from build123d import *

# Parameters (mm, degrees)
SKETCH_1_W              = 50
SKETCH_1_H              = 320
EXTRUDE_1_DEPTH         = 7.5
EXTRUDE_2_DEPTH         = 52.5
EXTRUDE_2_DEPTH_BACK    = 7.5
SKETCH_2_R              = 25
SKETCH_3_R              = 15
CUT_EXTRUDE_1_DEPTH     = 197.086715511
HOLE_WIZARD_12_0_12_1_D = 12


with BuildPart() as part:
    # 草图1 → 凸台-拉伸1 (new, symmetric)
    with BuildSketch(Plane(origin=(0, 0, 0), x_dir=(0, 0, -1), z_dir=(1, 0, 0))):
        Rectangle(SKETCH_1_W, SKETCH_1_H)
    extrude(amount=EXTRUDE_1_DEPTH, both=True)

    # 草图2 → 凸台-拉伸2 (add, two sides: drawn at the far end of the back side and taken through both)
    with BuildSketch(Plane(origin=(0, 0, 0), x_dir=(0, 0, -1), z_dir=(1, 0, 0)).offset(-EXTRUDE_2_DEPTH_BACK)):
        with Locations((0, 160)):
            Circle(SKETCH_2_R)
    extrude(amount=EXTRUDE_2_DEPTH + EXTRUDE_2_DEPTH_BACK)

    # 草图3 → 切除-拉伸1 (cut, through all)
    with BuildSketch(Plane(origin=(52.5, 0, 0), x_dir=(0, 0, -1), z_dir=(1, 0, 0))):
        with Locations((0, 160)):
            Circle(SKETCH_3_R)
    extrude(amount=-CUT_EXTRUDE_1_DEPTH, mode=Mode.SUBTRACT)

    # Ø12.0 (12) 直径孔1 (through all)
    with Locations(Plane.ZY.offset(7.5)):
        with Locations((0, 22), (0, -148)):
            Hole(HOLE_WIZARD_12_0_12_1_D / 2)


solid = part.part
The model under review builds one solid part; all positions refer to its coordinate system, in mm. A direction names the side the tool comes from. Round coordinates to 2 decimals unless told otherwise and drop trailing zeros. Write each loop counter-clockwise with the first axis right and the second up, starting at its lowest first coordinate (ties: lowest second). Pieces come first, ordered by that corner, then holes. Notation, with made-up numbers: M -16,86.25 L 3,86.25 A8 ccw 3,94.25 Z; hole C 63.5,-17.75 d6. An arc over 180 degrees is marked long. Answer as CSV lines item,"result". Start each with the question number.
Q1. Consider section A-A, the plane z = 0. Give the boundary of the cut face in (x, y).
Q2. Tool access review of faces 1 (the face through (22.08, 184.787, 3.255)), 2 (the face through (0.105, 16.143, 1.301)): name each direction out of +Z, -Z, +X, -X, +Y, -Y from which nothing blocks a thin tool from reaching the whole face with its end or side.
Q3. Clearance check with flat-ended pins moving along their axes: P1, Ø1, axis at x = 28, z = -3.5, coming from the +Y side; P2, Ø4, axis at y = 74, z = 8.5, coming from the +X side; P3, Ø5, axis at x = 22, z = -13.5, coming from the +Y side; P4, Ø15.5, axis at y = -148, z = 0, coming from the -X side. State where each tip first meets the part, or that it passes through.
Q4. Wall thickness on line 1 along Y through (x, z) = (0, 0); line 2 along Y through (x, z) = (11, 0); line 3 along X through (y, z) = (-6, 16): over which ranges is each line inside the solid? List them lowest first.
Q5. Consider section B-B, the plane y = 22. Give the boundary of the cut face in (x, z).
Q6. Consider section C-C, the plane x = 47. Give the boundary of the cut face in (y, z), then the cut area to 3 significant figures.
Q7. Consider section D-D, the plane z = -18.5. Give the boundary of the cut face in (x, y).
Q8. The part is to be moulded in two halves that separate along Y. For faces 3 (the face through (0, -160, 0)), 4 (the face through (0.105, -153.857, 1.301)), 5 (the face through (-7.5, 15, 0)), say which applies: +Y half, -Y half, draft (parallel to the pull), parting line (faces both ways), or undercut.
Result set:
1,outline,"M -7.5,-160 L 7.5,-160 L 7.5,-154 L -7.5,-154 Z; M -7.5,-142 L 7.5,-142 L 7.5,16 L -7.5,16 Z; M -7.5,28 L 7.5,28 L 7.5,135 L 52.5,135 L 52.5,145 L -7.5,145 Z; M -7.5,175 L 52.5,175 L 52.5,185 L -7.5,185 Z"
2,face 1,"+X"
2,face 2,"+X, -X"
3,P1,"stops at y = 184.82"
3,P2,"stops at x = 7.5"
3,P3,"stops at y = 182.45"
3,P4,"stops at x = -7.5"
4,line 1,"y = -160 to -154, -142 to 16, 28 to 145, 175 to 185"
4,line 2,"y = 135 to 145, 175 to 185"
4,line 3,"x = -7.5 to 7.5"
5,outline,"M -7.5,-25 L 7.5,-25 L 7.5,-6 L -7.5,-6 Z; M -7.5,6 L 7.5,6 L 7.5,25 L -7.5,25 Z"
6,outline,"C 160,0 d50; hole C 160,0 d30"
6,area,"1,260 mm²"
7,outline,"M -7.5,-160 L 7.5,-160 L 7.5,143.18 L 52.5,143.18 L 52.5,176.82 L -7.5,176.82 Z"
8,face 3,"-Y half"
8,face 4,"undercut"
8,face 5,"draft"
